Print and shaded views of the part. All mm, measured from the part's lowest x, y and z. A direction names the side the tool comes from. Round coordinates to 2 decimals unless told otherwise and drop trailing zeros. Order: outer loops, then holes, each group sorted by start corner. A loop starts at its lowest first (then second) coordinate and runs counter-clockwise, first axis right, second up. Notation, with made-up numbers: (78.5, 31.5) - (89.5, 31.5) arc R31 ccw to (89.5, 56.5) - close; hole circle Ø3 at (32.25, 22.25). An arc over 180 degrees is marked (long way). Write item = value, one per line. Start each with the question number.
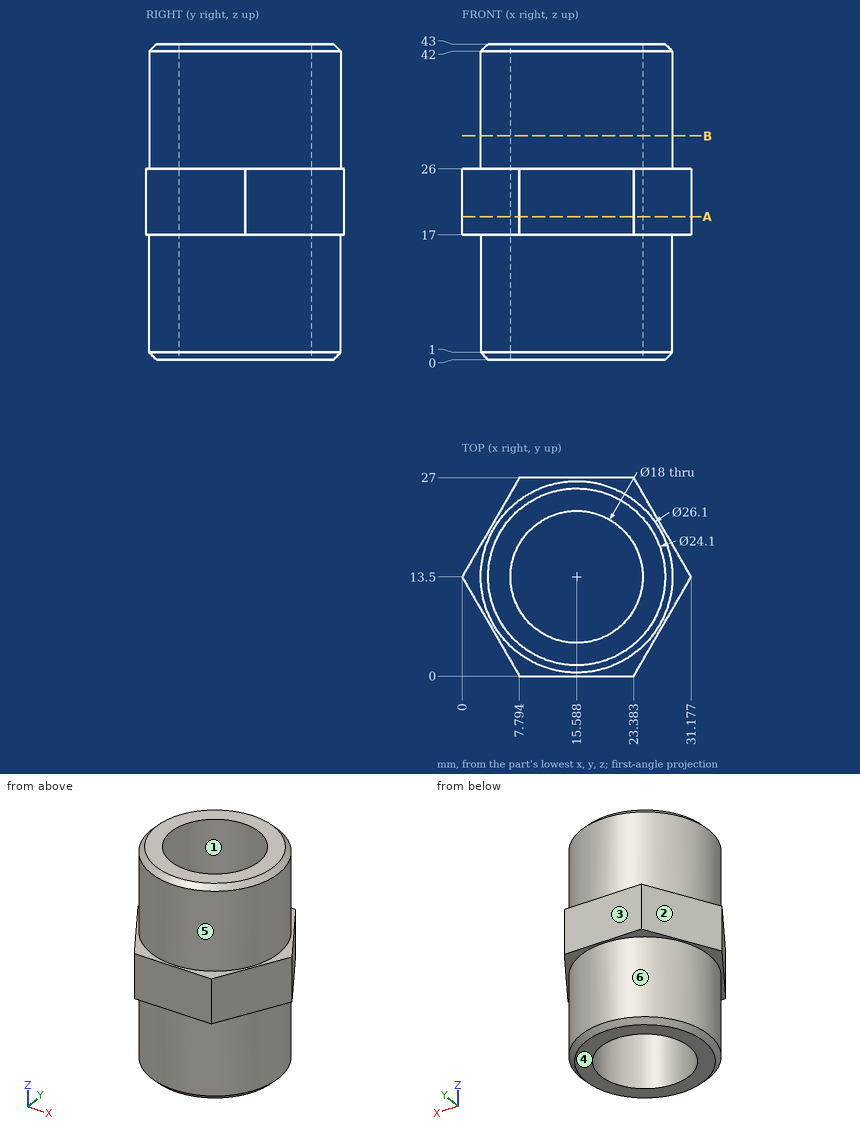
Item 1: Drop flat-ended pins along their axis: pin 1 (1.5 mm diameter, centred on y = 19.5, z = 23, fed in from +X) (1 decimal); pin 2 (1.5 mm diameter, centred on y = 11, z = 24.5, fed in from -X); pin 3 (1.5 mm diameter, centred on y = 22.5, z = 6.5, fed in from +X). Give the stop position or say it passes through.
Item 2: Mould opens along X. For the marked faces 1, 2 and 3 say: +X half, -X half, draft (parallel to the pull), parting line (faces both ways), or undercut.
Item 3: Saw through at B-B, the plane z = 30.5. Give the cut face in (x, y).
Item 4: Saw through at A-A, the plane z = 19.5. Give the cut face in (x, y) (1 decimal).
Item 5: Which spindle directions (+Z, -Z, +X, -X, +Y, -Y) get a long thin tool onto all of the face, cutting with end or side? Do the marked faces 4, 5 and 6. Say none if no direction does.
Item 6: Probe L1, parallel to Y at x = 11, z = 23; L2, parallel to Y at x = 8, z = 3 (1 decimal); L3, parallel to Z at x = 10, y = 25.75. List the from-to ranges inside material, lowest first.
Check sheet entries:
q1.pin_1 = 28.1
q1.pin_2 = 1.01
q1.pin_3 = 25.7
q2.face_1 = undercut
q2.face_2 = -X half
q2.face_3 = draft
q3.outline = circle Ø26.1 at (15.59, 13.5); hole circle Ø18 at (15.59, 13.5)
q4.outline = (0, 13.5) - (7.8, 0) - (23.4, 0) - (31.2, 13.5) - (23.4, 27) - (7.8, 27) - close; hole circle Ø18 at (15.6, 13.5)
q5.face_4 = -Z, +X, -X, +Y, -Y
q5.face_5 = +Z
q5.face_6 = -Z
q6.L1 = 0 to 5.76, 21.24 to 27
q6.L2 = 2.9 to 8.7, 18.3 to 24.1
q6.L3 = 17 to 26
